Geometry check sheet. Reference: the model listing, model coordinates, mm. A direction names the side the tool comes from. Coordinates: 2 decimals unless noted, no trailing zeros. Loops run counter-clockwise (first coordinate to the right, second up) from the corner with the lowest first, then second, coordinate; pieces in that order, holes last. Notation, with made-up numbers: (48, 26.25) - (86, 26.25) arc R22 cw to (86, 43.25) - close; hole circle Ø4 at (66, 46). An arc over 180 degrees is marked (long way). Write each question's results on one line, items separated by ' | '. Start each with the question number.
(1) Sectioned sample at C-C (z = 25). Enter the section's corners in (x, y), plus the area to 3 significant figures.
(2) Mould release check, pull along Y, two halves, no side actions. Record for faces 1 (the face through (55, 10, 25)), 2 (the face through (54, 20, 0)), 3 (the face through (55, 22, 10)): pulls with the +Y half, pulls with the -Y half, needs draft (parallel to the pull), parting line crosses it, or undercut.
(3) Sectioned sample at B-B (y = 35). Enter the section's corners in (x, z), plus the area to 3 significant figures.
(4) Access from +Z, -Z, +X, -X, +Y, -Y to the whole of each face (thin tool, end or side, straight path). Record for faces 4 (the face through (35, 0, 25)), 5 (the face through (15, 28, 25)), 6 (the face through (107, 5, 10)).
(5) Go/stop test with flat-tipped pins: pin 1 Ø6 at (y, z) = (59, 12) entering from +X; pin 2 Ø12 at (x, z) = (106, 15) entering from +Y; pin 3 Ø6 at (y, z) = (-2, 28) entering from -X; pin 4 Ø12 at (x, y) = (66.5, 1.5) entering from +Z. Record where each tip stops, or that it passes through.
(6) Sectioned sample at D-D (x = 55). Enter the section's corners in (y, z), plus the area to 3 significant figures.
(7) Material ranges on probe 1 along X at (y, z) = (35, 36); probe 2 along X at (y, z) = (52, 31.5); probe 3 along Z at (x, y) = (52, 61), recorded low to high.
(8) Sectioned sample at A-A (x = 17). Enter the section's corners in (y, z), plus the area to 3 significant figures.
from build123d import *

# Parameters (mm, degrees)
BASE_BODY_DEPTH          = 50
UPPER_BLOCK_DEPTH        = 50
CENTRE_START             = -10
CENTRE_WEB_DEPTH         = 10
FOOT_SLOT_1_DEPTH        = 7
FOOT_SLOT_2_DEPTH        = 7
BEARING_SEAT_CUT_1_DEPTH = 10
BEARING_START            = -10
BEARING_SEAT_CUT_2_DEPTH = 10


with BuildPart() as part:
    # Base Body Profile Sketch → Base Body (new body)
    with BuildSketch(Plane.XY):
        with BuildLine():
            Line((0, 0), (25, 0))
            Line((25, 0), (25, -10))
            Line((25, -10), (35, -10))
            Line((35, -10), (35, 10))
            Line((35, 10), (75, 10))
            Line((75, 10), (75, -10))
            Line((75, -10), (85, -10))
            Line((85, -10), (85, 0))
            Line((85, 0), (110, 0))
            Line((110, 0), (110, 10))
            Line((110, 10), (95, 10))
            Line((95, 10), (95, 55))
            Line((95, 55), (80, 55))
            Line((80, 55), (70, 65))
            Line((70, 65), (62.5, 65))
            Line((62.5, 65), (62.5, 48))
            Line((62.5, 48), (62.5, 45.618380291))
            ThreePointArc((62.5, 45.618380291), (55, 22), (47.5, 45.618380291))
            Line((47.5, 45.618380291), (47.5, 48))
            Line((47.5, 48), (47.5, 65))
            Line((47.5, 65), (40, 65))
            Line((40, 65), (30, 55))
            Line((30, 55), (15, 55))
            Line((15, 55), (15, 10))
            Line((15, 10), (0, 10))
            Line((0, 10), (0, 0))
        make_face()
    extrude(amount=BASE_BODY_DEPTH)

    # Upper Block Sketch → Upper Block (add)
    with BuildSketch(Plane(origin=(0, 65, 0), x_dir=(1, 0, 0), z_dir=(0, 1, 0))):
        Polygon((47.5, -20), (47.5, -25), (47.5, -30), (62.5, -30), (62.5, -20), align=None)
    extrude(amount=-UPPER_BLOCK_DEPTH)

    # Centre Web Sketch → Centre Web (add)
    with BuildSketch(Plane.XY.offset(30).offset(CENTRE_START)):
        with BuildLine():
            Line((47.5, 45.618380291), (47.5, 24.381619709))
            ThreePointArc((47.5, 24.381619709), (42, 35), (47.5, 45.618380291))
        make_face()
        with BuildLine():
            Line((62.5, 45.618380291), (62.5, 24.381619709))
            ThreePointArc((62.5, 24.381619709), (68, 35), (62.5, 45.618380291))
        make_face()
    extrude(amount=CENTRE_WEB_DEPTH)

    # Foot Slot 1 Sketch → Foot Slot 1 (cut)
    with BuildSketch(Plane.ZY):
        Polygon((25, 10), (10, 10), (10, 0), (40, 0), (40, 10), align=None)
    extrude(amount=-FOOT_SLOT_1_DEPTH, mode=Mode.SUBTRACT)

    # Foot Slot 2 Sketch → Foot Slot 2 (cut)
    with BuildSketch(Plane(origin=(110, 0, 0), x_dir=(0, 0, -1), z_dir=(1, 0, 0))):
        Polygon((-25, 10), (-40, 10), (-40, 0), (-10, 0), (-10, 10), align=None)
    extrude(amount=-FOOT_SLOT_2_DEPTH, mode=Mode.SUBTRACT)

    # Bearing Seat Cut 1 Sketch → Bearing Seat Cut 1 (cut)
    with BuildSketch(Plane(origin=(95, 0, 0), x_dir=(0, 0, -1), z_dir=(1, 0, 0))):
        with BuildLine():
            Line((-42, 55), (-8, 55))
            ThreePointArc((-8, 55), (-25, 38), (-42, 55))
        make_face()
    extrude(amount=-BEARING_SEAT_CUT_1_DEPTH, mode=Mode.SUBTRACT)

    # Bearing Seat Cut 2 Sketch → Bearing Seat Cut 2 (cut)
    with BuildSketch(Plane.ZY.offset(-15).offset(BEARING_START)):
        with BuildLine():
            Line((8, 55), (42, 55))
            ThreePointArc((42, 55), (25, 38), (8, 55))
        make_face()
    extrude(amount=BEARING_SEAT_CUT_2_DEPTH, mode=Mode.SUBTRACT)


solid = part.part
Outcome:
1) outline: (7, 0) - (25, 0) - (25, -10) - (35, -10) - (35, 10) - (75, 10) - (75, -10) - (85, -10) - (85, 0) - (103, 0) - (103, 10) - (95, 10) - (95, 38) - (85, 38) - (85, 55) - (80, 55) - (70, 65) - (40, 65) - (30, 55) - (25, 55) - (25, 38) - (15, 38) - (15, 10) - (7, 10) - close | area: 4,420 mm2
2) face 1: pulls with the -Y half | face 2: needs draft | face 3: undercut
3) outline: (15, 0) - (42, 0) - (42, 20) - (68, 20) - (68, 0) - (95, 0) - (95, 50) - (68, 50) - (68, 30) - (42, 30) - (42, 50) - (15, 50) - close | area: 2,960 mm2
4) face 4: +Z, -Z, -Y | face 5: +Z, -Z, -X, +Y | face 6: +X, +Y, -Y
5) pin 1: stops at x = 79 | pin 2: stops at y = 10 | pin 3: stops at x = 7 | pin 4: passes through
6) outline: (10, 0) - (22, 0) - (22, 20) - (65, 20) - (65, 30) - (22, 30) - (22, 50) - (10, 50) - close | area: 1,030 mm2
7) probe 1: x = 15 to 42, 68 to 95 | probe 2: x = 25 to 47.5, 62.5 to 85 | probe 3: z = 20 to 30
8) outline: (0, 0) - (55, 0) - (55, 8) arc R17 cw to (55, 42) - (55, 50) - (0, 50) - close | area: 2,300 mm2
